Here's how the part is built. I have some questions about the finished solid (model axes, mm). A direction names the side the tool comes from. Coordinates: 2 decimals unless noted, no trailing zeros. Order: outer loops, then holes, each group sorted by start corner. A loop starts at its lowest first (then second) coordinate and runs counter-clockwise, first axis right, second up. Notation, with made-up numbers: (58.25, -11.75) - (63.25, -11.75) arc R12 cw to (63.25, 7.25) - close; hole circle Ø9 at (-5, 85). An arc over 180 degrees is marked (long way). Answer in a Markdown table with one row per item. Add a question column.
Item 1: On a 3-axis mill with a long thin cutter (end or side, diameter ignored), from which of +Z, -Z, +X, -X, +Y, -Y can I reach the whole of each face in a straight line? I mean faces 1 (the flat face through (18, 25, -14)), 2 (the flat face through (10, 25, 6)), 3 (the cylindrical face through (-37.534, 7.535, -0.521)). Say none if no direction works.
Item 2: I want a section at B-B (x = 41.5). Please give me the cut outline in (y, z).
Item 3: I want a section at C-C (y = 13). Please give me the cut outline in (x, z), plus the area to 3 significant figures.
Item 4: Will these pins go through, and if not, where does the flat tip stop? pin 1 Ø5 at (x, y) = (-12, 18) entering from -Z; pin 2 Ø12 at (y, z) = (13, -1) entering from -X; pin 3 Ø8 at (x, y) = (-7, 25.5) entering from +Z; pin 4 Ø7 at (x, z) = (-41.5, 0) entering from +Y.
Item 5: I want a section at D-D (z = 0). Count the separate pieces of the cut face and the enclosed holes in it, plus the area to 4 significant figures.
Item 6: I want a section at A-A (y = 25). Please give me the cut outline in (x, z).
Item 7: If I drill on line 1 along X through (y, z) = (6.25, 0); line 2 along X through (y, z) = (2.25, 0); line 3 along Z through (x, y) = (18, 25), over which ranges is the centre line in solid material (lowest first)? Write a range as from..to.
Item 8: Thinking about a two-plate mould opening in Z: for faces 4 (the flat face through (17, 25, -7)), 5 (the flat face through (-47, 5, 0)), 6 (the flat face through (18, 25, 14)), which applies, +Z half, -Z half, draft (parallel to the pull), parting line (faces both ways), or undercut?
```python
from build123d import *

# Parameters (mm, degrees)
SKETCH1_W           = 94
SKETCH1_H           = 38
BOSS_EXTRUDE1_DEPTH = 10
SKETCH2_R           = 4
CUT_EXTRUDE1_DEPTH  = 5
SKETCH3_R           = 2.5
CUT_EXTRUDE2_DEPTH  = 5
SKETCH4_W           = 28
SKETCH4_H           = 30
BOSS_EXTRUDE2_DEPTH = 15
CUT_EXTRUDE3_DEPTH  = 109
CUT_EXTRUDE4_DEPTH  = 70


with BuildPart() as part:
    # Sketch1 → Boss-Extrude1 (new body)
    with BuildSketch(Plane(origin=(0, 0, 0), x_dir=(1, 0, 0), z_dir=(0, 1, 0))):
        Rectangle(SKETCH1_W, SKETCH1_H)
    extrude(amount=BOSS_EXTRUDE1_DEPTH)

    # Sketch2 → Cut-Extrude1 (cut)
    with BuildSketch(Plane(origin=(0, 10, 0), x_dir=(1, 0, 0), z_dir=(0, 1, 0))):
        with Locations(Location((-41.5, 0, 0), (0, 0, 270))):
            Circle(SKETCH2_R)
    cut_extrude1 = extrude(amount=-CUT_EXTRUDE1_DEPTH, mode=Mode.SUBTRACT)

    # Sketch3 → Cut-Extrude2 (cut)
    with BuildSketch(Plane(origin=(0, 5, 0), x_dir=(1, 0, 0), z_dir=(0, 1, 0))):
        with Locations(Location((-41.5, 0, 0), (0, 0, 270))):
            Circle(SKETCH3_R)
    cut_extrude2 = extrude(amount=-CUT_EXTRUDE2_DEPTH, mode=Mode.SUBTRACT)

    # Sketch4 → Boss-Extrude2 (add)
    with BuildSketch(Plane.ZY.offset(25)):
        with Locations((0, 25)):
            Rectangle(SKETCH4_W, SKETCH4_H)
    boss_extrude2 = extrude(amount=-BOSS_EXTRUDE2_DEPTH)

    # Sketch6 → Cut-Extrude3 (cut)
    with BuildSketch(Plane.ZY.offset(25)):
        with BuildLine():
            Line((-7, 27.1), (-4.81170448, 27.1))
            ThreePointArc((-4.81170448, 27.1), (5.25, 25), (-4.81170448, 22.9))
            Line((-4.81170448, 22.9), (-7, 22.9))
            Line((-7, 22.9), (-7, 27.1))
        make_face()
    extrude(amount=-CUT_EXTRUDE3_DEPTH, mode=Mode.SUBTRACT)

    # Mirror1: Cut-Extrude1, Cut-Extrude2, Boss-Extrude2 across plane
    add(cut_extrude1.mirror(Plane(origin=(0, 0, 0), x_dir=(0, 0, 1), z_dir=(1, 0, 0))), mode=Mode.SUBTRACT)
    add(cut_extrude2.mirror(Plane(origin=(0, 0, 0), x_dir=(0, 0, 1), z_dir=(1, 0, 0))), mode=Mode.SUBTRACT)
    add(boss_extrude2.mirror(Plane(origin=(0, 0, 0), x_dir=(0, 0, 1), z_dir=(1, 0, 0))))

    # Sketch7 → Cut-Extrude4 (cut)
    with BuildSketch(Plane.ZY.offset(-10)):
        with BuildLine():
            Line((-7, 22.9), (-4.81170448, 22.9))
            ThreePointArc((-4.81170448, 22.9), (5.25, 25), (-4.81170448, 27.1))
            Line((-4.81170448, 27.1), (-7, 27.1))
            Line((-7, 27.1), (-7, 22.9))
        make_face()
    extrude(amount=-CUT_EXTRUDE4_DEPTH, mode=Mode.SUBTRACT)


solid = part.part
```
Values follow:
| question | item | result |
|---|---|---|
| 1 | face 1 | -Z, +X, -X, +Y |
| 1 | face 2 | +Z, -Z, +Y |
| 1 | face 3 | +Y |
| 2 | outline | (0, -19) - (10, -19) - (10, -4) - (5, -4) - (5, -2.5) - (0, -2.5) - close; (0, 2.5) - (5, 2.5) - (5, 4) - (10, 4) - (10, 19) - (0, 19) - close |
| 3 | outline | (-25, -14) - (-10, -14) - (-10, 14) - (-25, 14) - close; (10, -14) - (25, -14) - (25, 14) - (10, 14) - close |
| 3 | area | 840 mm^2 |
| 4 | pin 1 | stops at z = -14 |
| 4 | pin 2 | stops at x = -47 |
| 4 | pin 3 | stops at z = 14 |
| 4 | pin 4 | stops at y = 5 |
| 5 | separate pieces | 5 |
| 5 | enclosed holes | 0 |
| 5 | area | 1,395 mm^2 |
| 6 | outline | (-25, -14) - (-10, -14) - (-10, -7) - (-25, -7) - close; (-25, 5.25) - (-10, 5.25) - (-10, 14) - (-25, 14) - close; (10, -14) - (25, -14) - (25, -7) - (10, -7) - close; (10, 5.25) - (25, 5.25) - (25, 14) - (10, 14) - close |
| 7 | line 1 | x = -47..-45.5, -37.5..37.5, 45.5..47 |
| 7 | line 2 | x = -47..-44, -39..39, 44..47 |
| 7 | line 3 | z = -14..-7, 5.25..14 |
| 8 | face 4 | undercut |
| 8 | face 5 | draft |
| 8 | face 6 | +Z half |
